CAD build for the part. Positions are in the model's coordinates, mm. Face numbers are marked on the shaded views. A direction names the side the tool comes from. Coordinates: 2 decimals unless noted, no trailing zeros. Loops run counter-clockwise (first coordinate to the right, second up) from the corner with the lowest first, then second, coordinate; pieces in that order, holes last. Notation, with made-up numbers: (26, 38) -> (46, 38) arc R24 ccw to (46, 76) -> close; hole circle Ø10 at (-27.5, 79.25). An arc over 180 degrees is marked (long way). Write each question's results on one line, items separated by ' | '.
from build123d import *

# Parameters (mm, degrees)
SKETCH1_W               = 80
SKETCH1_H               = 40
BOSS_EXTRUDE1_DEPTH     = 20
CUT_EXTRUDE1_DEPTH      = 49.989794856
CUT_EXTRUDE1_DEPTH_BACK = 49.989794856
SKETCH3_R               = 15
BOSS_EXTRUDE2_DEPTH     = 410


with BuildPart() as part:
    # Sketch1 → Boss-Extrude1 (new, symmetric)
    with BuildSketch(Plane(origin=(0, 0, 0), x_dir=(0, 0, -1), z_dir=(1, 0, 0))):
        Rectangle(SKETCH1_W, SKETCH1_H)
    extrude(amount=BOSS_EXTRUDE1_DEPTH, both=True)

    # Sketch2 → Cut-Extrude1 (cut, two sides: drawn at the far end of the back side and taken through both)
    with BuildSketch(Plane(origin=(0, 0, 0), x_dir=(0, 0, -1), z_dir=(1, 0, 0)).offset(-CUT_EXTRUDE1_DEPTH_BACK)):
        Polygon((-40, 20), (-20, -20), (-40, -20), align=None)
        Polygon((40, 20), (40, -20), (20, -20), align=None)
    extrude(amount=CUT_EXTRUDE1_DEPTH + CUT_EXTRUDE1_DEPTH_BACK, mode=Mode.SUBTRACT)

    # Sketch3 → Boss-Extrude2 (add)
    with BuildSketch(Plane.XZ.offset(20)):
        with Locations(Location((0, 0, 0), (0, 0, 90))):
            Circle(SKETCH3_R)
    extrude(amount=BOSS_EXTRUDE2_DEPTH)


solid = part.part
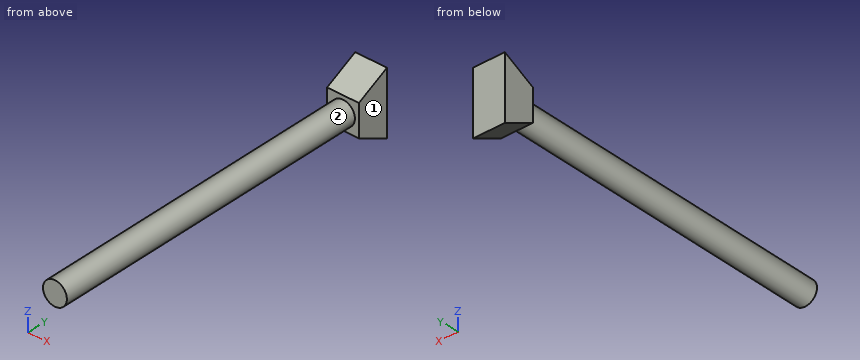
1) Slice it at C-C (y = -142). Write the cut outline in (x, z).
Outcome:
outline: circle Ø30 at (0, 0)
2) Slice it at D-D (y = -15.5). Write the cut outline in (x, z).
Outcome:
outline: (-20, -22.25) -> (20, -22.25) -> (20, 22.25) -> (-20, 22.25) -> close
3) Slice it at A-A (x = 0). Write the cut outline in (y, z).
Outcome:
outline: (-430, -15) -> (-20, -15) -> (-20, -20) -> (20, -40) -> (20, 40) -> (-20, 20) -> (-20, 15) -> (-430, 15) -> close
4) Pin check, flat tips, straight feed: pin 1 (10 mm diameter, centred on y = -233.5, z = -20.5, fed in from -X); pin 2 (5 mm diameter, centred on x = 5.5, z = -27, fed in from -Y); pin 3 (8 mm diameter, centred on x = 10, y = -221.5, fed in from -Z); pin 4 (4 mm diameter, centred on x = 12.5, y = -369.5, fed in from +Z). Stop position of each tip, or through.
Outcome:
pin 1: passes through | pin 2: stops at y = -11 | pin 3: stops at z = -13.75 | pin 4: stops at z = 10.71
5) Drill centre lines: L1, parallel to Z at x = -1, y = -289.5; L2, parallel to Y at x = -9.5, z = 18.5; L3, parallel to X at y = -307, z = 0.5. Where is each one in solid material? Low to high. Write a range as from..to.
Outcome:
L1: z = -14.97..14.97 | L2: y = -20..20 | L3: x = -14.99..14.99
6) Which spindle directions (+Z, -Z, +X, -X, +Y, -Y) get a long thin tool onto all of the face, cutting with end or side? Do the marked faces 1 and 2. Say none if no direction does.
Outcome:
face 1: +Z, -Z, +X, +Y, -Y | face 2: -Y
7) Slice it at B-B (z = 0). Write the cut outline in (x, y).
Outcome:
outline: (-20, -20) -> (-15, -20) -> (-15, -430) -> (15, -430) -> (15, -20) -> (20, -20) -> (20, 20) -> (-20, 20) -> close
